```python
from build123d import *

# Parameters (mm, degrees)
GB_6728_1986_050_X_50_X_3_1_DEPTH = 695


with BuildPart() as part:
    # Sketch1 → Gb／6728-1986方形空心型钢 050 X 50 X 3(1) (new body)
    with BuildSketch(Plane.YX.offset(-347.5)):
        with BuildLine():
            Line((-19, -25), (19, -25))
            ThreePointArc((19, -25), (23.242640687, -23.242640687), (25, -19))
            Line((25, -19), (25, 19))
            ThreePointArc((25, 19), (23.242640687, 23.242640687), (19, 25))
            Line((19, 25), (-19, 25))
            ThreePointArc((-19, 25), (-23.242640687, 23.242640687), (-25, 19))
            Line((-25, 19), (-25, -19))
            ThreePointArc((-25, -19), (-23.242640687, -23.242640687), (-19, -25))
        make_face()
        with BuildLine():
            Line((-19, -22), (19, -22))
            ThreePointArc((19, -22), (21.121320344, -21.121320344), (22, -19))
            Line((22, -19), (22, 19))
            ThreePointArc((22, 19), (21.121320344, 21.121320344), (19, 22))
            Line((19, 22), (-19, 22))
            ThreePointArc((-19, 22), (-21.121320344, 21.121320344), (-22, 19))
            Line((-22, 19), (-22, -19))
            ThreePointArc((-22, -19), (-21.121320344, -21.121320344), (-19, -22))
        make_face(mode=Mode.SUBTRACT)
    extrude(amount=GB_6728_1986_050_X_50_X_3_1_DEPTH)


solid = part.part
```
Input: part model. Units: mm. Frame: model coordinates. A direction names the side the tool comes from. Give positions to 0.01 mm unless a question says otherwise; leave off trailing zeros. Order: outer loops, then holes, each group sorted by start corner. A loop starts at its lowest first (then second) coordinate and runs counter-clockwise, first axis right, second up.
1. Mould query, pull axis X, two halves, no side actions, for faces 3 (the flat face through (0.1, -22.3, 347.5)), 4 (the flat face through (25, 0, 5)), 5 (the flat face through (0, -22, 5)). Classes: released by +X, released by -X, zero draft, split by the parting line, or undercut.
Derived:
face 3: zero draft
face 4: released by +X
face 5: undercut
2. Section C-C on z = 286.5. Return the cut outline in (x, y).
Derived:
outline: (-25, -19) arc R6 ccw to (-19, -25) - (19, -25) arc R6 ccw to (25, -19) - (25, 19) arc R6 ccw to (19, 25) - (-19, 25) arc R6 ccw to (-25, 19) - close; hole (-22, -19) arc R3 ccw to (-19, -22) - (19, -22) arc R3 ccw to (22, -19) - (22, 19) arc R3 ccw to (19, 22) - (-19, 22) arc R3 ccw to (-22, 19) - close
3. Reachability of faces 1 (the flat face through (-25, 0, 5)), 2 (the flat face through (0, 22, 5)) from +Z, -Z, +X, -X, +Y, -Y: full face, straight path, thin tool, end or side. Return the list, or none.
Derived:
face 1: +Z, -Z, -X, +Y, -Y
face 2: +Z, -Z
4. Section A-A on y = 7. Return the cut outline in (x, z), and give its area (3 significant figures).
Derived:
outline: (-25, -347.5) - (-22, -347.5) - (-22, 347.5) - (-25, 347.5) - close; (22, -347.5) - (25, -347.5) - (25, 347.5) - (22, 347.5) - close
area: 4,170 mm2
5. Material intervals for L1, parallel to Y at x = 11.5, z = -228; L2, parallel to X at y = -20, z = 91, sorted ascending.
Derived:
L1: y = -25 to -22, 22 to 25
L2: x = -24.92 to -21.83, 21.83 to 24.92
